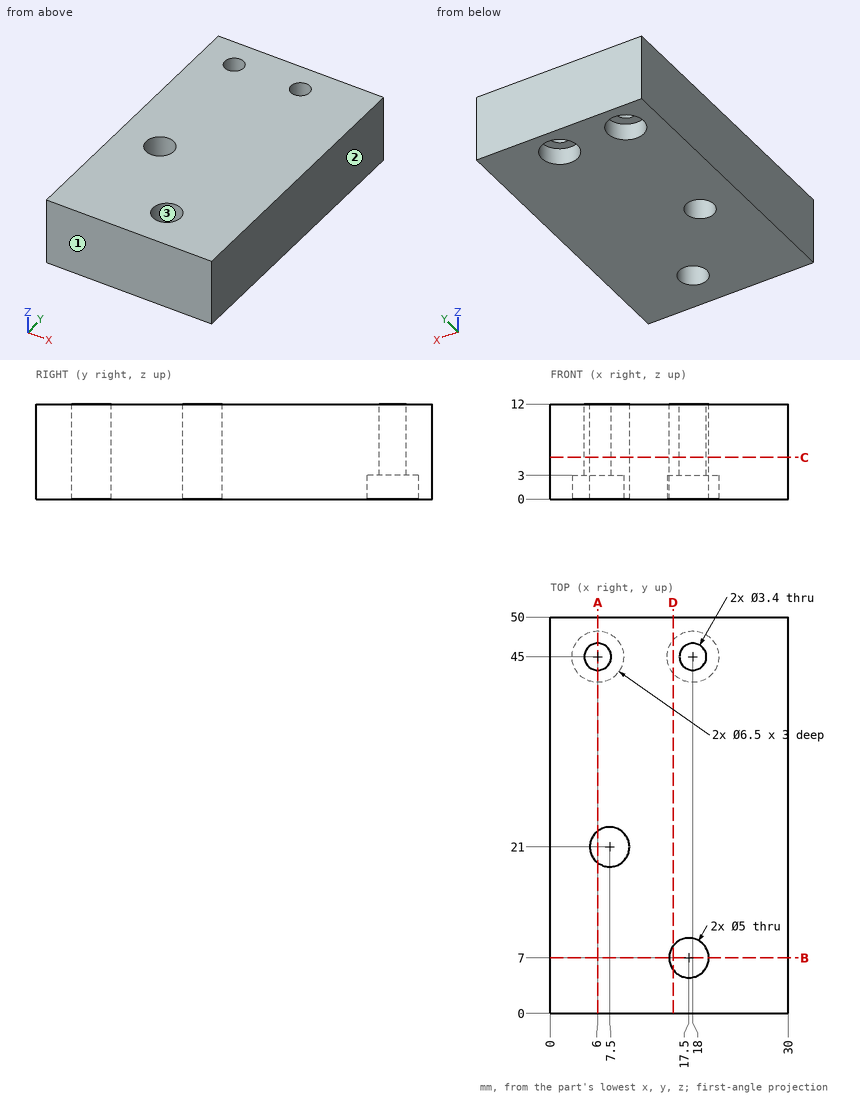
Drawing for the job (mm, zero at the part's lowest x, y, z). Coordinates: 2 decimals unless noted, no trailing zeros. Order: outer loops, then holes, each group sorted by start corner. A loop starts at its lowest first (then second) coordinate and runs counter-clockwise, first axis right, second up. Notation, with made-up numbers: (-34, 36.5) -> (-10, 36.5) arc R19 cw to (-10, 47.5) -> close; hole circle Ø6 at (-15.5, -15). An arc over 180 degrees is marked (long way). One line per item, written item: value.
(1) Mould opens along X. For the marked faces 1, 2 and 3 say: pulls with the +X half, pulls with the -X half, needs draft (parallel to the pull), parting line crosses it, or undercut.
Checked values:
face 1: needs draft
face 2: pulls with the +X half
face 3: undercut
(2) Slice it at C-C, the plane z = 5.25. List the corners of the cut face in (x, y), plus the area to 3 significant figures.
Checked values:
outline: (0, 0) -> (30, 0) -> (30, 50) -> (0, 50) -> close; hole circle Ø3.4 at (6, 45); hole circle Ø5 at (7.5, 21); hole circle Ø5 at (17.5, 7); hole circle Ø3.4 at (18, 45)
area: 1,440 mm2
(3) Probe line 1 (Y direction, x = 6, z = 1); line 2 (Y direction, x = 18, z = 1.8); line 3 (X direction, y = 6.5, z = 11). List the from-to ranges inside material, lowest first. Write a range as [from, to].
Checked values:
line 1: [0, 19], [23, 41.75], [48.25, 50]
line 2: [0, 4.55], [9.45, 41.75], [48.25, 50]
line 3: [0, 15.05], [19.95, 30]
(4) Slice it at B-B, the plane y = 7. List the corners of the cut face in (x, z).
Checked values:
outline: (0, 0) -> (15, 0) -> (15, 12) -> (0, 12) -> close; (20, 0) -> (30, 0) -> (30, 12) -> (20, 12) -> close
(5) Slice it at D-D, the plane x = 15.5. List the corners of the cut face in (y, z), plus the area to 3 significant figures.
Checked values:
outline: (0, 0) -> (5.5, 0) -> (5.5, 12) -> (0, 12) -> close; (8.5, 0) -> (42.92, 0) -> (42.92, 3) -> (47.08, 3) -> (47.08, 0) -> (50, 0) -> (50, 12) -> (8.5, 12) -> close
area: 552 mm2
(6) Slice it at A-A, the plane x = 6. List the corners of the cut face in (y, z), plus the area to 3 significant figures.
Checked values:
outline: (0, 0) -> (19, 0) -> (19, 12) -> (0, 12) -> close; (23, 0) -> (41.75, 0) -> (41.75, 3) -> (43.3, 3) -> (43.3, 12) -> (23, 12) -> close; (46.7, 3) -> (48.25, 3) -> (48.25, 0) -> (50, 0) -> (50, 12) -> (46.7, 12) -> close
area: 502 mm2
(7) Drop a flat-ended pin along its axis: pin 1 Ø5 at (x, y) = (6, 45) entering from -Z. Give the stop position or say it passes through.
Checked values:
pin 1: z = 3
